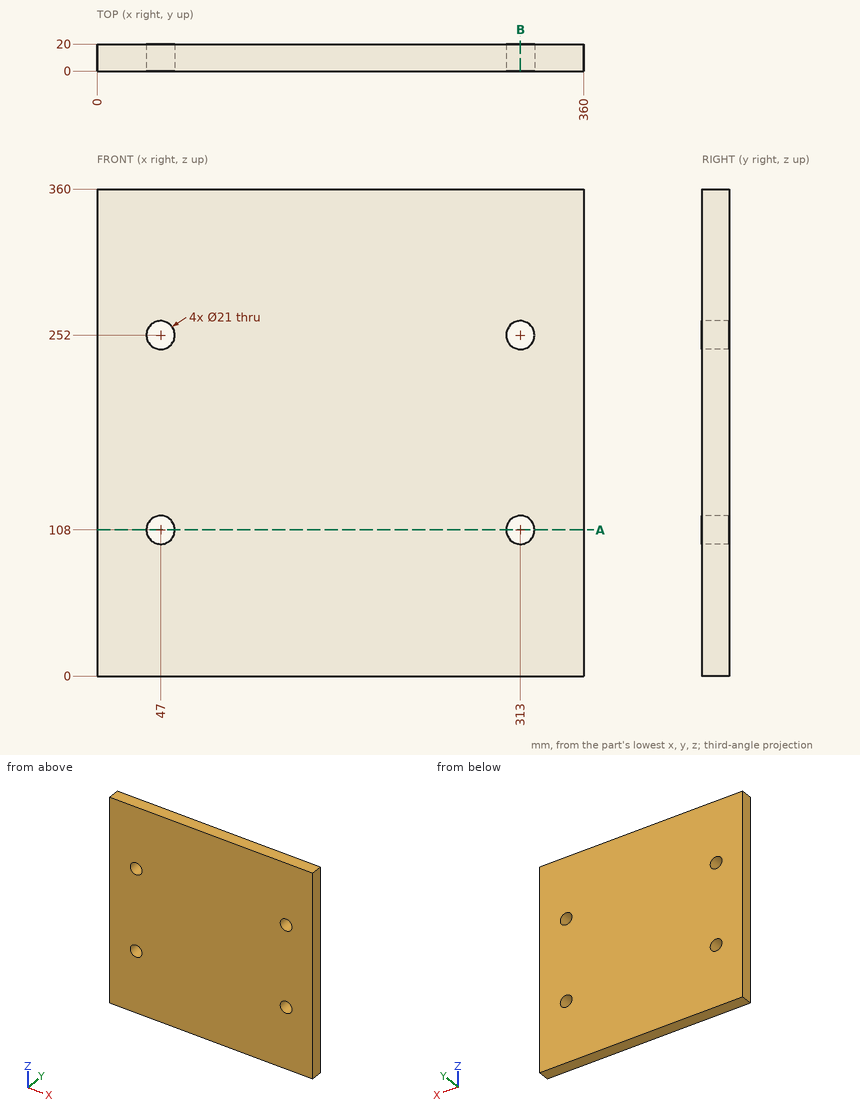
Study the drawing (mm; zero at the part's minimum x, y, z) and answer. Round coordinates to 2 decimals unless told otherwise and drop trailing zeros. Order: outer loops, then holes, each group sorted by start corner. A loop starts at its lowest first (then second) coordinate and runs counter-clockwise, first axis right, second up. Notation, with made-up numbers: M 40.25,-15 L 89.25,-15 A30 ccw 89.25,7 Z; hole C 60,67 d5. An arc over 180 degrees is marked long. One line per item, written item: value.
Q1. A flat-ended cylindrical pin translates along its axis: pin 1 (17 mm diameter, centred on x = 313, z = 252, fed in from -Y). Find the tip coordinate at first contact, or state that the pin passes through.
Derived:
pin 1: through
Q2. Straight lines are drawn through the part: line 1 (Z direction, x = 313, y = 11); line 2 (Z direction, x = 53, y = 1). For each, find the intervals that lie inside material, in ascending order.
Derived:
line 1: 0 to 97.5, 118.5 to 241.5, 262.5 to 360
line 2: 0 to 99.38, 116.62 to 243.38, 260.62 to 360
Q3. Find section A-A on z = 108. Write down the section's boundary in (x, y), then the cut area to 3 significant figures.
Derived:
outline: M 0,0 L 36.5,0 L 36.5,20 L 0,20 Z; M 57.5,0 L 302.5,0 L 302.5,20 L 57.5,20 Z; M 323.5,0 L 360,0 L 360,20 L 323.5,20 Z
area: 6,360 mm²
Q4. Find section B-B on x = 313. Write down the section's boundary in (y, z).
Derived:
outline: M 0,0 L 20,0 L 20,97.5 L 0,97.5 Z; M 0,118.5 L 20,118.5 L 20,241.5 L 0,241.5 Z; M 0,262.5 L 20,262.5 L 20,360 L 0,360 Z
